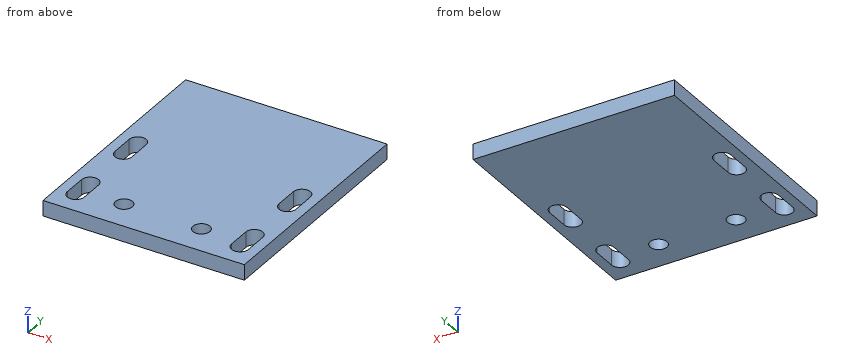
from build123d import *

# Parameters (mm, degrees)
SKETCH1_W                  = 130
SKETCH1_H                  = 130
BOSS_EXTRUDE1_DEPTH        = 10
F_11_0_11_DIAMETER_HOLE1_D = 11
SKETCH4_W                  = 130
SKETCH4_H                  = 10
BOSS_EXTRUDE2_DEPTH        = 20
M6_CLEARANCE_HOLE1_D       = 7
CUT_EXTRUDE1_DEPTH         = 199.746069144


with BuildPart() as part:
    # Sketch1 → Boss-Extrude1 (new body)
    with BuildSketch(Plane.XY):
        with Locations((65, 65)):
            Rectangle(SKETCH1_W, SKETCH1_H)
    extrude(amount=BOSS_EXTRUDE1_DEPTH)

    # Ø11.0 (11) Diameter Hole1 (through all)
    with Locations(Plane.XY.offset(10)):
        with Locations((40, 20), (90, 20)):
            Hole(F_11_0_11_DIAMETER_HOLE1_D / 2)

    # Sketch4 → Boss-Extrude2 (add)
    with BuildSketch(Plane(origin=(0, 130, 0), x_dir=(1, 0, 0), z_dir=(0, 1, 0))):
        with Locations((65, -5)):
            Rectangle(SKETCH4_W, SKETCH4_H)
    extrude(amount=BOSS_EXTRUDE2_DEPTH)

    # M6 Clearance Hole1 (through all)
    with Locations(Plane(origin=(0, 0, 0), x_dir=(-1, 0, 0), z_dir=(0, 0, -1))):
        with Locations((-118, 68.5), (-118, 18.5), (-12, 68.5), (-12, 18.5)):
            Hole(M6_CLEARANCE_HOLE1_D / 2)

    # Sketch8 → Cut-Extrude1 (cut, through all)
    with BuildSketch(Plane(origin=(0, 0, 0), x_dir=(-1, 0, 0), z_dir=(0, 0, -1))):
        with BuildLine():
            Line((-123.5, 15), (-123.5, 30))
            ThreePointArc((-123.5, 30), (-118, 35.5), (-112.5, 30))
            Line((-112.5, 30), (-112.5, 15))
            ThreePointArc((-112.5, 15), (-118, 9.5), (-123.5, 15))
        make_face()
        with BuildLine():
            Line((-123.5, 65), (-123.5, 80))
            ThreePointArc((-123.5, 80), (-118, 85.5), (-112.5, 80))
            Line((-112.5, 80), (-112.5, 65))
            ThreePointArc((-112.5, 65), (-118, 59.5), (-123.5, 65))
        make_face()
        with BuildLine():
            Line((-17.5, 65), (-17.5, 80))
            ThreePointArc((-17.5, 80), (-12, 85.5), (-6.5, 80))
            Line((-6.5, 80), (-6.5, 65))
            ThreePointArc((-6.5, 65), (-12, 59.5), (-17.5, 65))
        make_face()
        with BuildLine():
            Line((-17.5, 15), (-17.5, 30))
            ThreePointArc((-17.5, 30), (-12, 35.5), (-6.5, 30))
            Line((-6.5, 30), (-6.5, 15))
            ThreePointArc((-6.5, 15), (-12, 9.5), (-17.5, 15))
        make_face()
    extrude(amount=-CUT_EXTRUDE1_DEPTH, mode=Mode.SUBTRACT)


solid = part.part
Input: part model. Units: mm. Frame: model coordinates. Round coordinates to 2 decimals unless told otherwise and drop trailing zeros. Order: outer loops, then holes, each group sorted by start corner. A loop starts at its lowest first (then second) coordinate and runs counter-clockwise, first axis right, second up.
1. Material intervals for line 1 (X direction, y = 30, z = 3.5); line 2 (Y direction, x = 12.5, z = 6); line 3 (Y direction, x = 90, z = 4), sorted ascending.
The answers:
line 1: x = 0 to 6.5, 17.5 to 112.5, 123.5 to 130
line 2: y = 0 to 9.52, 35.48 to 59.52, 85.48 to 150
line 3: y = 0 to 14.5, 25.5 to 150
2. Pin query (flat end, axial travel): P1, Ø10, axis at x = 40, y = 20, coming from the -Z side. Return the tip coordinate at first contact, or that it passes through.
The answers:
P1: passes through
3. Cut plane C-C, the plane x = 118. Output: boundary loops of the cut face in (y, z), then the cut area to 3 significant figures.
The answers:
outline: (0, 0) - (9.5, 0) - (9.5, 10) - (0, 10) - close; (35.5, 0) - (59.5, 0) - (59.5, 10) - (35.5, 10) - close; (85.5, 0) - (150, 0) - (150, 10) - (85.5, 10) - close
area: 980 mm2
4. Cut plane A-A, the plane x = 90. Output: boundary loops of the cut face in (y, z).
The answers:
outline: (0, 0) - (14.5, 0) - (14.5, 10) - (0, 10) - close; (25.5, 0) - (150, 0) - (150, 10) - (25.5, 10) - close
5. Cut plane D-D, the plane y = 20. Output: boundary loops of the cut face in (x, z), then the cut area to 3 significant figures.
The answers:
outline: (0, 0) - (6.5, 0) - (6.5, 10) - (0, 10) - close; (17.5, 0) - (34.5, 0) - (34.5, 10) - (17.5, 10) - close; (45.5, 0) - (84.5, 0) - (84.5, 10) - (45.5, 10) - close; (95.5, 0) - (112.5, 0) - (112.5, 10) - (95.5, 10) - close; (123.5, 0) - (130, 0) - (130, 10) - (123.5, 10) - close
area: 860 mm2
6. Cut plane B-B, the plane y = 72. Output: boundary loops of the cut face in (x, z).
The answers:
outline: (0, 0) - (6.5, 0) - (6.5, 10) - (0, 10) - close; (17.5, 0) - (112.5, 0) - (112.5, 10) - (17.5, 10) - close; (123.5, 0) - (130, 0) - (130, 10) - (123.5, 10) - close
